Geometry check sheet. Reference: the model listing, model coordinates, mm. Give positions to 0.01 mm unless a question says otherwise; leave off trailing zeros. Order: outer loops, then holes, each group sorted by start corner. A loop starts at its lowest first (then second) coordinate and runs counter-clockwise, first axis right, second up.
from build123d import *

# Parameters (mm, degrees)
EXTRUDE1_DEPTH          = 5
CUT_EXTRUDE1_DEPTH      = 8.5
CUT_EXTRUDE1_DEPTH_BACK = 8.5
FILLET2_R               = 0.25


with BuildPart() as part:
    # Sketch1 → Extrude1 (new body)
    with BuildSketch(Plane.XY):
        with BuildLine():
            Line((-2.5, 2.5), (2.5, 2.5))
            ThreePointArc((2.5, 2.5), (5, 0), (2.5, -2.5))
            Line((2.5, -2.5), (-2.5, -2.5))
            ThreePointArc((-2.5, -2.5), (-5, 0), (-2.5, 2.5))
        make_face()
    extrude(amount=EXTRUDE1_DEPTH)

    # Sketch2 → Cut-Extrude1 (cut, two sides: drawn at the far end of the back side and taken through both)
    with BuildSketch(Plane(origin=(0, 0, 0), x_dir=(1, 0, 0), z_dir=(0, 1, 0)).offset(-CUT_EXTRUDE1_DEPTH_BACK)):
        Polygon((-5, 0), (5, 0), (5, -0.1), align=None)
    extrude(amount=CUT_EXTRUDE1_DEPTH + CUT_EXTRUDE1_DEPTH_BACK, mode=Mode.SUBTRACT)

    # Fillet2
    fillet2_edges = [part.edges().sort_by_distance(p)[0] for p in [
        (5, 0, 5),
        (0, 2.5, 5),
        (-4.267744857, -1.767789049, 0.007322551),
        (0, -2.5, 0.05),
        (4.267744857, -1.767789049, 0.092677449),
        (0, 2.5, 0.05),
        (-5, 0, 5),
        (0, -2.5, 5),
    ]]
    fillet(fillet2_edges, radius=FILLET2_R)


solid = part.part
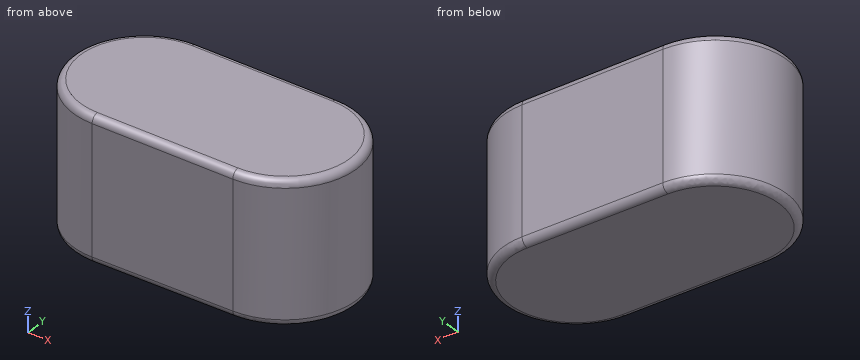
Item 1: Scan lines: L1, parallel to Z at x = 2.75, y = -1.75; L2, parallel to Z at x = -2.75, y = 2.25; L3, parallel to X at y = -1.75, z = 3.3. Record each from-to range of solid material in increasing order.
Reported:
L1: z = 0.08 to 5
L2: z = 0.02 to 5
L3: x = -4.29 to 4.29
Item 2: Gauge pin test, flat ends, axial feed: pin 1 (2 mm diameter, centred on x = 3.5, y = 0.5, fed in from -Z) (3 decimals); pin 2 (1 mm diameter, centred on y = 1, z = 1, fed in from +X). Record the tip position at first contact, or that the pin passes through.
Reported:
pin 1: stops at z = 0.075
pin 2: stops at x = 4.95
Item 3: Sectioned sample at A-A (z = 1.65). Enter the section's corners in (x, y), and give its area (3 significant figures).
Reported:
outline: (-2.5, -2.5) - (2.5, -2.5) arc R2.5 ccw to (2.5, 2.5) - (-2.5, 2.5) arc R2.5 ccw to start
area: 44.6 mm2
